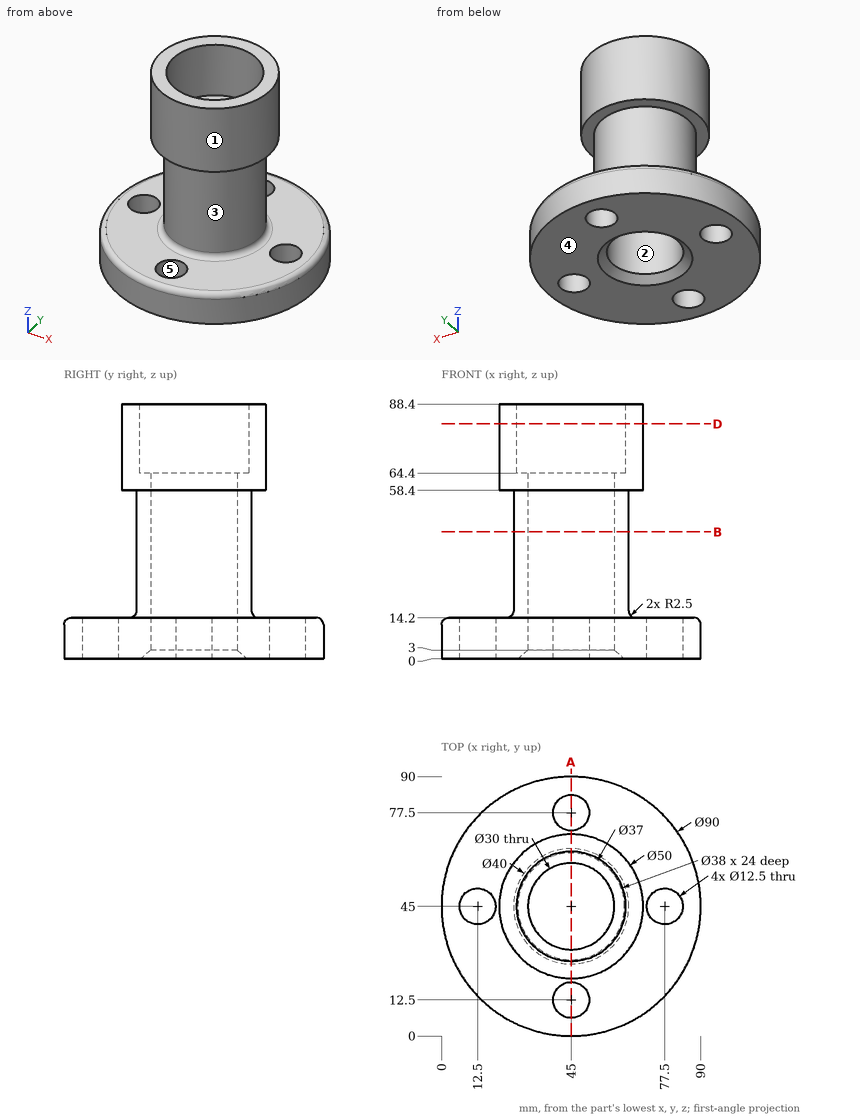
Geometry: see drawing. Coordinates: mm, zero at the bounding-box minimum. A direction names the side the tool comes from. Round coordinates to 2 decimals unless told otherwise and drop trailing zeros. Loops run counter-clockwise (first coordinate to the right, second up) from the corner with the lowest first, then second, coordinate; pieces in that order, holes last. Notation, with made-up numbers: M -19.75,74.5 L 22.25,74.5 A19 ccw 22.25,98.5 Z; hole C 1,39 d7. An arc over 180 degrees is marked long. Use a Markdown table: item, result. Add a question column.
1. Reachability of the marked faces 1 and 2 from +Z, -Z, +X, -X, +Y, -Y: full face, straight path, thin tool, end or side. Return the list, or none.
2. Section query B-B on z = 44. Return the cut outline in (x, y), then the cut area to 3 significant figures.
3. Mould query, pull axis Z, two halves, no side actions, for the marked faces 3, 4 and 5. Classes: pulls with the +Z half, pulls with the -Z half, needs draft (parallel to the pull), parting line crosses it, or undercut.
4. Contact query for flat-ended pins moving along their axis: P1, Ø4, axis at x = 14.5, y = 67, coming from the +Z side; P2, Ø6, axis at y = 66, z = 70.5, coming from the +X side; P3, Ø1.5, axis at x = 59, y = 52.5, coming from the -Z side; P4, Ø10, axis at x = 31.5, y = 23.5, coming from the -Z side. Output: stop coordinate, or through.
5. Line query: line 1 (X direction, y = 44, z = 4); line 2 (Y direction, x = 45, z = 70.5); line 3 (Z direction, x = 51, y = 68). Output: solid intervals per line, ascending.
6. Section query D-D on z = 81.5. Return the cut outline in (x, y).
7. Section query A-A on x = 45. Give the number of separate pieces and of enclosed holes in the cut face, then the cut area to 3 significant figures.
Reported:
| question | item | result |
|---|---|---|
| 1 | face 1 | +Z |
| 1 | face 2 | +Z, -Z |
| 2 | outline | C 45,45 d40; hole C 45,45 d30 |
| 2 | area | 550 mm² |
| 3 | face 3 | undercut |
| 3 | face 4 | pulls with the -Z half |
| 3 | face 5 | needs draft |
| 4 | P1 | stops at z = 14.2 |
| 4 | P2 | stops at x = 62.35 |
| 4 | P3 | stops at z = 1.6 |
| 4 | P4 | stops at z = 0 |
| 5 | line 1 | x = 0.01 to 6.33, 18.67 to 30.03, 59.97 to 71.33, 83.67 to 89.99 |
| 5 | line 2 | y = 20 to 26, 64 to 70 |
| 5 | line 3 | z = 0 to 14.2, 58.4 to 88.4 |
| 6 | outline | C 45,45 d50; hole C 45,45 d38 |
| 7 | separate pieces | 4 |
| 7 | enclosed holes | 0 |
| 7 | area | 1,340 mm² |
